Source: CAD feature listing. Evaluate the final solid. Frame: model axes, mm. Round coordinates to 2 decimals unless told otherwise and drop trailing zeros. Loops run counter-clockwise (first coordinate to the right, second up) from the corner with the lowest first, then second, coordinate; pieces in that order, holes last. Notation, with made-up numbers: (-9, -39) - (25, -39) arc R18 ccw to (25, -8) - close; hole circle Ø6 at (40.5, 48). An arc over 180 degrees is marked (long way). Use CSV: the item, a comma, the result in double quotes. Start each with the question number.
from build123d import *

# Parameters (mm, degrees)
SKETCH_1_W              = 169
SKETCH_1_H              = 279
EXTRUDE_1_DEPTH         = 2.5
HOLE_WIZARD_5_5_5_5_1_D = 5.5
CHAMFER_1_SIZE          = 5


with BuildPart() as part:
    # 草图1 → 凸台-拉伸1 (new, symmetric)
    with BuildSketch(Plane(origin=(0, 0, 0), x_dir=(1, 0, 0), z_dir=(0, 1, 0))):
        Rectangle(SKETCH_1_W, SKETCH_1_H)
    extrude(amount=EXTRUDE_1_DEPTH, both=True)

    # Ø5.5 (5.5) 直径孔1 (through all)
    with Locations(Plane(origin=(0, -2.5, 0), x_dir=(-1, 0, 0), z_dir=(0, -1, 0))):
        with Locations((75, -130), (-75, -130), (-75, 130), (75, 130)):
            Hole(HOLE_WIZARD_5_5_5_5_1_D / 2)

    # 倒角1
    chamfer_1_edges = [part.edges().sort_by_distance(p)[0] for p in [
        (-84.5, 0, -139.5),
        (84.5, 0, -139.5),
        (84.5, 0, 139.5),
        (-84.5, 0, 139.5),
    ]]
    chamfer(chamfer_1_edges, length=CHAMFER_1_SIZE)


solid = part.part
1. Section query B-B on z = 130. Return the cut outline in (x, y), and give its area (3 significant figures).
2. Mould query, pull axis X, two halves, no side actions, for faces 1 (the flat face through (82, 0, 137)), 2 (the cylindrical face through (-77.182, 0.035, -128.327)), 3 (the cylindrical face through (72.818, 0.035, 131.673)), 4 (the flat face through (-82, 0, 137)). Classes: +X half, -X half, draft (parallel to the pull), parting line (faces both ways), or undercut.
3. Section query A-A on x = 75. Return the cut outline in (y, z), and give its area (3 significant figures).
4. Line query: line 1 along X through (y, z) = (-0.25, -130); line 2 along Z through (x, y) = (75, 1.1); line 3 along Z through (x, y) = (-77, 1.3). Output: solid intervals per line, ascending.
Values:
1,outline,"(-84.5, -2.5) - (-77.75, -2.5) - (-77.75, 2.5) - (-84.5, 2.5) - close; (-72.25, -2.5) - (72.25, -2.5) - (72.25, 2.5) - (-72.25, 2.5) - close; (77.75, -2.5) - (84.5, -2.5) - (84.5, 2.5) - (77.75, 2.5) - close"
1,area,"790 mm^2"
2,face 1,"+X half"
2,face 2,"undercut"
2,face 3,"undercut"
2,face 4,"-X half"
3,outline,"(-2.5, -139.5) - (2.5, -139.5) - (2.5, -132.75) - (-2.5, -132.75) - close; (-2.5, -127.25) - (2.5, -127.25) - (2.5, 127.25) - (-2.5, 127.25) - close; (-2.5, 132.75) - (2.5, 132.75) - (2.5, 139.5) - (-2.5, 139.5) - close"
3,area,"1,340 mm^2"
4,line 1,"x = -84.5 to -77.75, -72.25 to 72.25, 77.75 to 84.5"
4,line 2,"z = -139.5 to -132.75, -127.25 to 127.25, 132.75 to 139.5"
4,line 3,"z = -139.5 to -131.89, -128.11 to 128.11, 131.89 to 139.5"
